from build123d import *

# Parameters (mm, degrees)
SKETCH_1_W             = 80
SKETCH_1_H             = 120
SKETCH_1_W_2           = 76
SKETCH_1_H_2           = 116
EXTRUDE_1_DEPTH        = 350
CUT_EXTRUDE_2_REACH    = 366.005
SKETCH_4_R             = 25
HOLE_WIZARD_M4_1_D     = 3.3
HOLE_WIZARD_M4_1_DEPTH = 2
HOLE_WIZARD_M3_1_D     = 3.6
HOLE_WIZARD_M3_1_DEPTH = 2
CUT_EXTRUDE_3_REACH    = 374.156
SKETCH_16_W            = 50
SKETCH_16_H            = 30
SKETCH_16_W_2          = 60
SKETCH_16_H_2          = 100
FILLET_1_R             = 6


with BuildPart() as part:
    # 草图1 → 拉伸-薄壁1 (new, symmetric)
    with BuildSketch(Plane.XY):
        Rectangle(SKETCH_1_W, SKETCH_1_H)
        Rectangle(SKETCH_1_W_2, SKETCH_1_H_2, mode=Mode.SUBTRACT)
    extrude(amount=EXTRUDE_1_DEPTH, both=True)

    # 草图4 → 切除-拉伸2 (cut, up to next)
    with BuildSketch(Plane.ZY.offset(40), mode=Mode.PRIVATE) as cut_extrude_2_sk1:
        with Locations((0, -20)):
            Circle(SKETCH_4_R)
    cut_extrude_2_tool1 = extrude(cut_extrude_2_sk1.sketch, amount=-CUT_EXTRUDE_2_REACH, mode=Mode.PRIVATE) & part.part
    add(cut_extrude_2_tool1.solids().sort_by_distance((-40, -20, 0))[0], mode=Mode.SUBTRACT)

    # Hole Wizard M4 _1
    with Locations(Plane.ZY.offset(40)):
        with Locations((304.5, 29), (304.5, 15), (304.5, 7), (304.5, -7), (-304.5, -7), (-304.5, 7), (-304.5, 15), (-304.5, 29)):
            Hole(HOLE_WIZARD_M4_1_D / 2, depth=HOLE_WIZARD_M4_1_DEPTH)

    # M3 间隙孔1
    with Locations(Plane(origin=(0, 60, 0), x_dir=(1, 0, 0), z_dir=(0, 1, 0))):
        with Locations((-17.5, 345), (20.5, 345), (20.5, 99), (-17.5, 99), (-20.5, -345), (17.5, -345), (-20.5, -99), (17.5, -99)):
            Hole(HOLE_WIZARD_M3_1_D / 2, depth=HOLE_WIZARD_M3_1_DEPTH)

    # 草图16 → 切除-拉伸3 (cut, up to next)
    with BuildSketch(Plane.XZ.offset(60), mode=Mode.PRIVATE) as cut_extrude_3_sk1:
        with Locations((0, 330)):
            Rectangle(SKETCH_16_W, SKETCH_16_H)
    cut_extrude_3_tool1 = extrude(cut_extrude_3_sk1.sketch, amount=-CUT_EXTRUDE_3_REACH, mode=Mode.PRIVATE) & part.part
    # 草图16 → 切除-拉伸3 (cut, up to next)
    with BuildSketch(Plane.XZ.offset(60), mode=Mode.PRIVATE) as cut_extrude_3_sk2:
        with Locations((0, 145)):
            Rectangle(SKETCH_16_W_2, SKETCH_16_H_2)
    cut_extrude_3_tool2 = extrude(cut_extrude_3_sk2.sketch, amount=-CUT_EXTRUDE_3_REACH, mode=Mode.PRIVATE) & part.part
    # 草图16 → 切除-拉伸3 (cut, up to next)
    with BuildSketch(Plane.XZ.offset(60), mode=Mode.PRIVATE) as cut_extrude_3_sk3:
        with Locations((0, -145)):
            Rectangle(SKETCH_16_W_2, SKETCH_16_H_2)
    cut_extrude_3_tool3 = extrude(cut_extrude_3_sk3.sketch, amount=-CUT_EXTRUDE_3_REACH, mode=Mode.PRIVATE) & part.part
    # 草图16 → 切除-拉伸3 (cut, up to next)
    with BuildSketch(Plane.XZ.offset(60), mode=Mode.PRIVATE) as cut_extrude_3_sk4:
        with Locations((0, -330)):
            Rectangle(SKETCH_16_W, SKETCH_16_H)
    cut_extrude_3_tool4 = extrude(cut_extrude_3_sk4.sketch, amount=-CUT_EXTRUDE_3_REACH, mode=Mode.PRIVATE) & part.part
    add(cut_extrude_3_tool1.solids().sort_by_distance((0, -60, 330))[0], mode=Mode.SUBTRACT)
    add(cut_extrude_3_tool2.solids().sort_by_distance((0, -60, 145))[0], mode=Mode.SUBTRACT)
    add(cut_extrude_3_tool3.solids().sort_by_distance((0, -60, -145))[0], mode=Mode.SUBTRACT)
    add(cut_extrude_3_tool4.solids().sort_by_distance((0, -60, -330))[0], mode=Mode.SUBTRACT)

    # 圆角1
    fillet_1_edges = [part.edges().sort_by_distance(p)[0] for p in [
        (25, -59, 315),
        (25, -59, 345),
        (-25, -59, 345),
        (-25, -59, 315),
        (30, -59, 95),
        (30, -59, 195),
        (-30, -59, 195),
        (-30, -59, 95),
        (30, -59, -95),
        (-30, -59, -95),
        (-30, -59, -195),
        (30, -59, -195),
        (25, -59, -315),
        (-25, -59, -315),
        (-25, -59, -345),
        (25, -59, -345),
    ]]
    fillet(fillet_1_edges, radius=FILLET_1_R)


solid = part.part
Source: CAD feature listing. Evaluate the final solid. Frame: model axes, mm. A direction names the side the tool comes from. Give positions to 0.01 mm unless a question says otherwise; leave off trailing zeros. Write each loop counter-clockwise with the first axis right and the second up, starting at its lowest first coordinate (ties: lowest second). Pieces come first, ordered by that corner, then holes. Notation, with made-up numbers: M 25.25,44.25 L 74.25,44.25 A21 cw 74.25,49.25 Z; hole C -31.5,75 d11. An arc over 180 degrees is marked long. Return JSON: item names as keys, results as strings. Group by question number.
1) Material intervals for line 1 along Z through (x, y) = (-20.5, 58.6); line 2 along X through (y, z) = (59, 99); line 3 along X through (y, z) = (-39, 139.5), sorted ascending. Write a range as [from, to].
2) Pull-direction query (X, two-part tool) for faces 4 (the face through (38.3, 18.1, 350)), 5 (the face through (-1, 58, 5)), 6 (the face through (40, -1, 5)), 7 (the face through (-40, 12, 5)); classes: pulls with the +X half, pulls with the -X half, needs draft (parallel to the pull), parting line crosses it, or undercut.
3) Cut plane C-C, the plane z = -63. Output: boundary loops of the cut face in (x, y), plus the area to 3 significant figures.
4) Pin query (flat end, axial travel): P1, Ø6, axis at x = -17.5, z = -99, coming from the -Y side; P2, Ø4, axis at y = 7, z = 304.5, coming from the -X side; P3, Ø2, axis at y = 29, z = -304.5, coming from the -X side. Return the tip coordinate at first contact, or that it passes through.
5) Cut plane A-A, the plane y = 47. Output: boundary loops of the cut face in (x, z), plus the area to 3 significant figures.
6) Set-up query: faces 1 (the face through (-39.014, -12.491, 23.846)), 2 (the face through (38.3, 18.1, -350)), 3 (the face through (-1, -58, 5)). Return all of +Z, -Z, +X, -X, +Y, -Y with unobstructed straight access to the full face (end or side cutting, diameter ignored); none if empty.
7) Cut plane B-B, the plane z = -154. Output: boundary loops of the cut face in (x, y), plus the area to 3 significant figures.
Recorded:
{
 "1": {"line 1": "z = [-350, 97.2], [100.8, 343.2], [346.8, 350]", "line 2": "x = [-40, -22.3], [-18.7, 15.7], [19.3, 40]", "line 3": "x = [-40, -38], [38, 40]"},
 "2": {"face 4": "needs draft", "face 5": "undercut", "face 6": "pulls with the +X half", "face 7": "pulls with the -X half"},
 "3": {"outline": "M -40,-60 L 40,-60 L 40,60 L -40,60 Z; hole M -38,-58 L 38,-58 L 38,58 L -38,58 Z", "area": "784 mm²"},
 "4": {"P1": "stops at y = 58", "P2": "stops at x = -40", "P3": "stops at x = 38"},
 "5": {"outline": "M -40,-350 L -38,-350 L -38,350 L -40,350 Z; M 38,-350 L 40,-350 L 40,350 L 38,350 Z", "area": "2,800 mm²"},
 "6": {"face 1": "-X", "face 2": "-Z, +X, -X, +Y, -Y", "face 3": "+Z, -Z"},
 "7": {"outline": "M -40,-60 L -30,-60 L -30,-58 L -38,-58 L -38,58 L 38,58 L 38,-58 L 30,-58 L 30,-60 L 40,-60 L 40,60 L -40,60 Z", "area": "664 mm²"}
}
